from build123d import *

# Parameters (mm, degrees)
SKETCH_1_R          = 3
EXTRUDE_1_DEPTH     = 5
SKETCH_3_R          = 6
CUT_EXTRUDE_1_DEPTH = 10
EXTRUDE_START       = -5
SKETCH_4_R          = 9
SKETCH_4_R_2        = 4.5
EXTRUDE_3_DEPTH     = 5


with BuildPart() as part:
    # 草图1 → 凸台-拉伸1 (new body)
    with BuildSketch(Plane.XY):
        with BuildLine():
            Line((0, 9), (120, 9))
            ThreePointArc((120, 9), (129, 0), (120, -9))
            Line((120, -9), (0, -9))
            ThreePointArc((0, -9), (-9, 0), (0, 9))
        make_face()
        Circle(SKETCH_1_R, mode=Mode.SUBTRACT)
        with Locations((120, 0)):
            Circle(SKETCH_1_R, mode=Mode.SUBTRACT)
    extrude(amount=EXTRUDE_1_DEPTH)

    # 草图3 → 切除-拉伸1 (cut)
    with BuildSketch(Plane.XY.offset(5)):
        with Locations((120, 0)):
            Circle(SKETCH_3_R)
    extrude(amount=-CUT_EXTRUDE_1_DEPTH, mode=Mode.SUBTRACT)

    # 草图4 → 凸台-拉伸3 (add)
    with BuildSketch(Plane.XY.offset(5).offset(EXTRUDE_START)):
        with Locations((120, 0)):
            Circle(SKETCH_4_R)
        with Locations((120, 0)):
            Circle(SKETCH_4_R_2, mode=Mode.SUBTRACT)
    extrude(amount=EXTRUDE_3_DEPTH)


solid = part.part
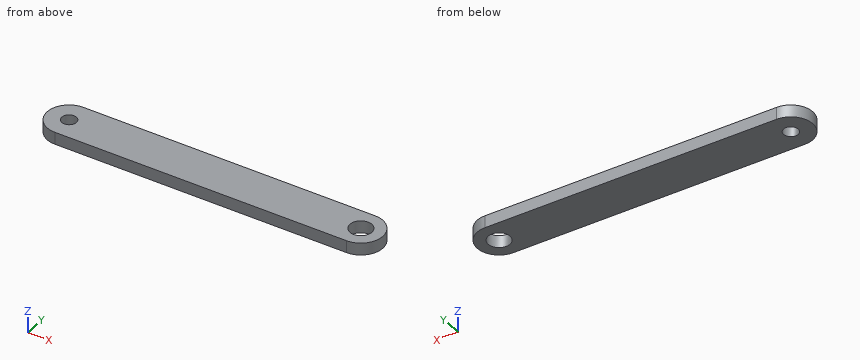
Design review of the part built by this model. Coordinates are the model's own, in mm. Coordinates: 2 decimals unless noted, no trailing zeros. Order: outer loops, then holes, each group sorted by start corner. A loop starts at its lowest first (then second) coordinate and runs counter-clockwise, first axis right, second up.
Item 1: Take a section at B-B, the plane z = 3.25. Write out the cut boundary in (x, y), then the cut area to 3 significant figures.
Item 2: Take a section at A-A, the plane y = 0. Write out the cut boundary in (x, z).
Item 3: For line 1 (Y direction, x = 120, z = 2.8); line 2 (X direction, y = 0.5, z = 3.7); line 3 (X direction, y = -0.75, z = 3.65), list the stretches that pass through material, from the lowest coordinate up.
Item 4: Take a section at C-C, the plane y = -6.5. Write out the cut boundary in (x, z).
The answers:
1. outline: (0, -9) - (120, -9) arc R9 ccw to (120, 9) - (0, 9) arc R9 ccw to start; hole circle Ø6 at (0, 0); hole circle Ø9 at (120, 0)
1. area: 2,320 mm2
2. outline: (-9, 0) - (-3, 0) - (-3, 5) - (-9, 5) - close; (3, 0) - (115.5, 0) - (115.5, 5) - (3, 5) - close; (124.5, 0) - (129, 0) - (129, 5) - (124.5, 5) - close
3. line 1: y = -9 to -4.5, 4.5 to 9
3. line 2: x = -8.99 to -2.96, 2.96 to 115.53, 124.47 to 128.99
3. line 3: x = -8.97 to -2.9, 2.9 to 115.56, 124.44 to 128.97
4. outline: (-6.22, 0) - (126.22, 0) - (126.22, 5) - (-6.22, 5) - close
